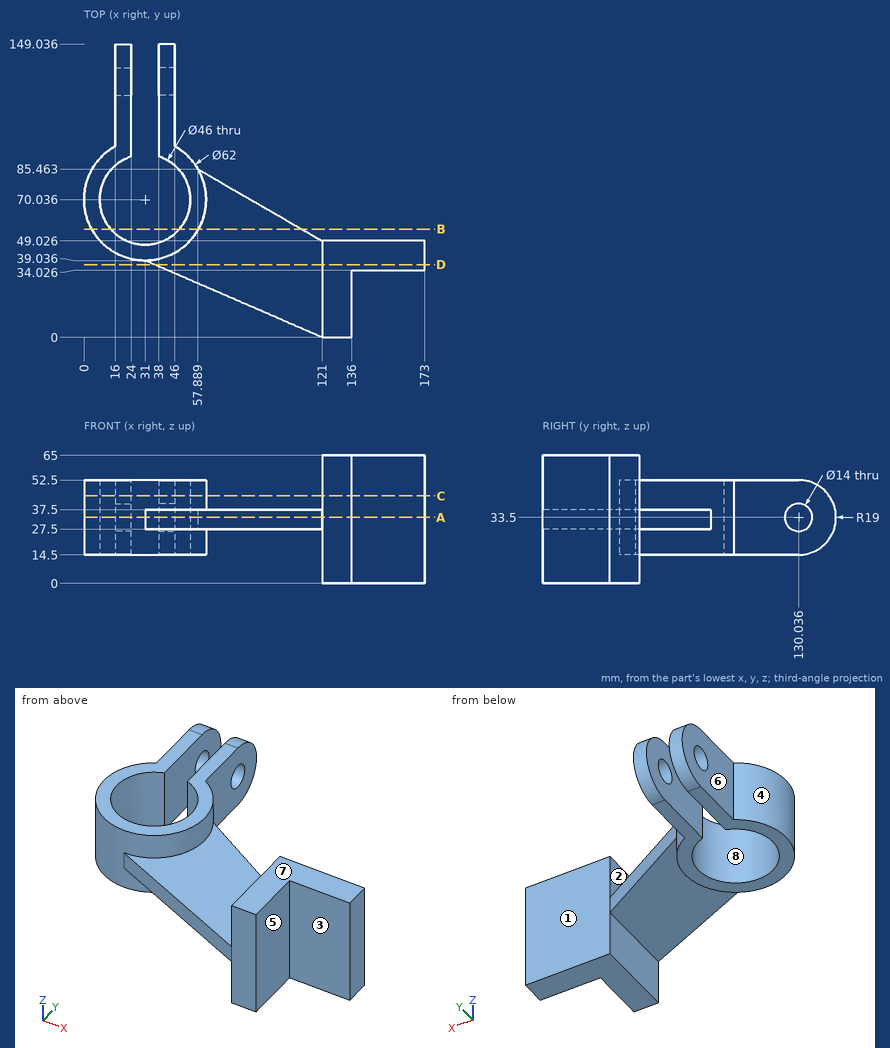
Print and shaded views of the part. All mm, measured from the part's lowest x, y and z. A direction names the side the tool comes from. Coordinates: 2 decimals unless noted, no trailing zeros. Loops run counter-clockwise (first coordinate to the right, second up) from the corner with the lowest first, then second, coordinate; pieces in that order, holes last. Notation, with made-up numbers: (21.25, 74) -> (61.25, 74) arc R21 cw to (61.25, 84) -> close; hole circle Ø7 at (39.5, 80). An arc over 180 degrees is marked (long way). Use a Markdown table: item, result. Add a question column.
Item 1: Which spindle directions (+Z, -Z, +X, -X, +Y, -Y) get a long thin tool onto all of the face, cutting with end or side? Do the marked faces 1, 2, 3 and 4. Say none if no direction does.
Item 2: Probe probe 1 along X at (y, z) = (98, 34); probe 2 along Y at (x, z) = (18.5, 33.5) (1 decimal); probe 3 along Y at (x, z) = (42.25, 33.5) (1 decimal). List the from-to ranges inside material, lowest first.
Item 3: Pull direction X, two halves, no side cores. Call the marked faces 5, 6, 7 and 8: +X half, -X half, draft (parallel to the pull), parting line (faces both ways), or undercut.
Item 4: Band-saw the part on A-A on z = 33.5. Write the cut outline in (x, y) (1 decimal).
Item 5: Band-saw the part on B-B on y = 55. Write the cut outline in (x, z) (1 decimal), plus the area to 3 significant figures.
Item 6: Band-saw the part on D-D on y = 37. Write the cut outline in (x, z) (1 decimal).
Item 7: Flat gauge pins, fed straight in: P1, Ø1, axis at y = 76, z = 39.5, coming from the -X side (1 decimal); P2, Ø15.5, axis at x = 155, z = 18, coming from the +Y side; P3, Ø10, axis at y = 65.5, z = 55.5, coming from the -X side (1 decimal). Where does each tip first touch, or does it go through?
Item 8: Band-saw the part on C-C on z = 44.5. Write the cut outline in (x, y) (1 decimal), plus the area to 3 significant figures.
Geometry says:
| question | item | result |
|---|---|---|
| 1 | face 1 | +Z, -Z, +X, +Y |
| 1 | face 2 | +Z, +Y, -Y |
| 1 | face 3 | +Z, -Z, +X, -Y |
| 1 | face 4 | none |
| 2 | probe 1 | 16 to 24, 38 to 46 |
| 2 | probe 2 | 41.7 to 50.7, 89.3 to 123, 137 to 149 |
| 2 | probe 3 | 34.2 to 50, 90.1 to 123, 137 to 149 |
| 3 | face 5 | +X half |
| 3 | face 6 | -X half |
| 3 | face 7 | draft |
| 3 | face 8 | undercut |
| 4 | outline | (16, 97.2) arc R31 ccw to (31, 39) -> (121, 0) -> (136, 0) -> (136, 34) -> (173, 34) -> (173, 49) -> (121, 49) -> (57.9, 85.5) arc R31 ccw to (46, 97.2) -> (46, 123) -> (38, 123) -> (38, 91.9) arc R23 cw (long way) to (24, 91.9) -> (24, 123) -> (16, 123) -> close; (16, 137) -> (24, 137) -> (24, 149) -> (16, 149) -> close; (38, 137) -> (46, 137) -> (46, 149) -> (38, 149) -> close |
| 5 | outline | (3.9, 14.5) -> (13.6, 14.5) -> (13.6, 52.5) -> (3.9, 52.5) -> close; (48.4, 14.5) -> (58.1, 14.5) -> (58.1, 27.5) -> (110.7, 27.5) -> (110.7, 37.5) -> (58.1, 37.5) -> (58.1, 52.5) -> (48.4, 52.5) -> close |
| 5 | area | 1,260 mm² |
| 6 | outline | (35.7, 27.5) -> (121, 27.5) -> (121, 0) -> (173, 0) -> (173, 65) -> (121, 65) -> (121, 37.5) -> (35.7, 37.5) -> close |
| 7 | P1 | x = 0.5 |
| 7 | P2 | y = 49.03 |
| 7 | P3 | x = 0 |
| 8 | outline | (16, 97.2) arc R31 ccw (long way) to (46, 97.2) -> (46, 145.5) -> (38, 145.5) -> (38, 91.9) arc R23 cw (long way) to (24, 91.9) -> (24, 145.5) -> (16, 145.5) -> close; (121, 0) -> (136, 0) -> (136, 34) -> (173, 34) -> (173, 49) -> (121, 49) -> close |
| 8 | area | 3,280 mm² |
